Could you check a few things on this model? Use its own coordinates, in mm. Coordinates: 2 decimals unless noted, no trailing zeros. Loops run counter-clockwise (first coordinate to the right, second up) from the corner with the lowest first, then second, coordinate; pieces in that order, holes last.
1) Will this pin go through, and if not, where does the flat tip stop? P1, Ø5.5, axis at x = 100, y = 145, coming from the -Z side.
2) Imagine slicing it at C-C on x = -108. Please give me the cut outline in (y, z), plus the area to 3 significant figures.
3) Thinking about a two-plate mould opening in X: for faces 1 (the face through (-3, 2, 4)), 2 (the face through (108.55, -79.006, 2.028)), which applies, released by +X, released by -X, zero draft, split by the parting line, or undercut?
4) Imagine slicing it at B-B on y = -88. Please give me the cut outline in (x, z), plus the area to 3 significant figures.
5) Imagine slicing it at A-A on z = 1.05. Please give me the cut outline in (x, y).
6) If I drill on line 1 along Y through (x, z) = (-199, 1.6); line 2 along X through (y, z) = (-91, 1.05); line 3 along X through (y, z) = (-84, 2.85), over which ranges is the centre line in solid material (lowest first)?
```python
from build123d import *

# Parameters (mm, degrees)
SKETCH_1_W          = 416
SKETCH_1_H          = 308
EXTRUDE_1_DEPTH     = 4
FILLET_1_R          = 2
CUT_EXTRUDE_1_REACH = 260.836
FILLET_2_R          = 2
HOLE_WIZARD_M6_1_D  = 7
HOLE_WIZARD_M6_2_D  = 7


with BuildPart() as part:
    # 草图1 → 凸台-拉伸1 (new body)
    with BuildSketch(Plane.XY):
        Rectangle(SKETCH_1_W, SKETCH_1_H)
    extrude(amount=EXTRUDE_1_DEPTH)

    # 圆角1
    fillet_1_edges = [part.edges().sort_by_distance(p)[0] for p in [
        (-208, 154, 2),
        (208, 154, 2),
        (208, -154, 2),
        (-208, -154, 2),
    ]]
    fillet(fillet_1_edges, radius=FILLET_1_R)

    # 草图2 → 切除-拉伸1 (cut, up to next)
    with BuildSketch(Plane.XY.offset(4), mode=Mode.PRIVATE) as cut_extrude_1_sk1:
        with BuildLine():
            Line((-133, -154), (-133, -104))
            ThreePointArc((-133, -104), (-108, -79), (-83, -104))
            Line((-83, -104), (-83, -154))
            ThreePointArc((-83, -154), (-108, -179), (-133, -154))
        make_face()
    cut_extrude_1_tool1 = extrude(cut_extrude_1_sk1.sketch, amount=-CUT_EXTRUDE_1_REACH, mode=Mode.PRIVATE) & part.part
    cut_extrude_1 = cut_extrude_1_tool1.solids().sort_by_distance((-108, -129, 4))[0]
    add(cut_extrude_1, mode=Mode.SUBTRACT)

    # 镜向1: 切除-拉伸1 across plane
    add(cut_extrude_1.mirror(Plane(origin=(0, 0, 0), x_dir=(0, 0, 1), z_dir=(1, 0, 0))), mode=Mode.SUBTRACT)

    # 圆角2
    fillet_2_edges = [part.edges().sort_by_distance(p)[0] for p in [
        (-133, -154, 2),
        (-83, -154, 2),
        (83, -154, 2),
        (133, -154, 2),
    ]]
    fillet(fillet_2_edges, radius=FILLET_2_R)

    # M6 间隙孔1 (through all)
    with Locations(Plane.XY.offset(4)):
        with Locations((-199, 80), (-199, -80)):
            hole_wizard_m6_1 = Hole(HOLE_WIZARD_M6_1_D / 2)

    # 镜向2: M6 间隙孔1 across plane
    add(hole_wizard_m6_1.mirror(Plane(origin=(0, 0, 0), x_dir=(0, 0, 1), z_dir=(1, 0, 0))), mode=Mode.SUBTRACT)

    # M6 间隙孔2 (through all)
    with Locations(Plane.XY.offset(4)):
        with Locations((-100, 145), (100, 145)):
            Hole(HOLE_WIZARD_M6_2_D / 2)


solid = part.part
```
Filled in:
1. P1: passes through
2. outline: (-79, 0) - (154, 0) - (154, 4) - (-79, 4) - close
2. area: 932 mm2
3. face 1: zero draft
3. face 2: undercut
4. outline: (-208, 0) - (-127.21, 0) - (-127.21, 4) - (-208, 4) - close; (-88.79, 0) - (88.79, 0) - (88.79, 4) - (-88.79, 4) - close; (127.21, 0) - (208, 0) - (208, 4) - (127.21, 4) - close
4. area: 1,360 mm2
5. outline: (-208, -152) arc R2 ccw to (-206, -154) - (-135, -154) arc R2 ccw to (-133, -152) - (-133, -104) arc R25 cw to (-83, -104) - (-83, -152) arc R2 ccw to (-81, -154) - (81, -154) arc R2 ccw to (83, -152) - (83, -104) arc R25 cw to (133, -104) - (133, -152) arc R2 ccw to (135, -154) - (206, -154) arc R2 ccw to (208, -152) - (208, 152) arc R2 ccw to (206, 154) - (-206, 154) arc R2 ccw to (-208, 152) - close; hole circle Ø7 at (-199, -80); hole circle Ø7 at (-199, 80); hole circle Ø7 at (-100, 145); hole circle Ø7 at (100, 145); hole circle Ø7 at (199, -80); hole circle Ø7 at (199, 80)
6. line 1: y = -154 to -83.5, -76.5 to 76.5, 83.5 to 154
6. line 2: x = -208 to -129.35, -86.65 to 86.65, 129.35 to 208
6. line 3: x = -208 to -123, -93 to 93, 123 to 208
